Design review of the part built by this model. Coordinates are the model's own, in mm. A direction names the side the tool comes from. Coordinates: 2 decimals unless noted, no trailing zeros. Order: outer loops, then holes, each group sorted by start corner. A loop starts at its lowest first (then second) coordinate and runs counter-clockwise, first axis right, second up. Notation, with made-up numbers: M 16.5,-31 L 31.5,-31 A16 cw 31.5,-1 Z; hole C 73.25,25.5 d8. An arc over 180 degrees is marked long. Answer as a JSON object with one key per item and string values.
from build123d import *


with BuildPart() as part:
    # Sketch1 → Revolve1 (revolve)
    with BuildSketch(Plane.XY, mode=Mode.PRIVATE) as revolve1_sk:
        Polygon((-20, 7), (-20, 5), (20, 5), (20, 6), (-15, 6), (-15, 5.9), (-16, 5.9), (-16, 7), align=None)
    revolve(revolve1_sk.sketch.rotate(Axis((20, 0, 0), (-1, 0, 0)), 270), axis=Axis((20, 0, 0), (-1, 0, 0)))


solid = part.part
1) Insertion check: pin 1 Ø1 at (y, z) = (4.5, -1) entering from -X; pin 2 Ø2 at (x, z) = (-1.5, -4) entering from +Y; pin 3 Ø6 at (x, y) = (11.5, 3.5) entering from +Z; pin 4 Ø1.5 at (x, y) = (-0.5, -2.5) entering from -Z. Each pin has a flat end and moves straight along its axis. Give the tip position at first contact, or say it passes through.
Taken from the geometry:
{"pin 1": "stops at x = -20", "pin 2": "stops at y = 5.2", "pin 3": "stops at z = 5.98", "pin 4": "stops at z = -5.74"}
2) Add section C-C (z = 5.5). State the section outline as (x, y) points, and give its area (3 significant figures).
Taken from the geometry:
{"outline": "M -20,-4.33 L -16,-4.33 L -16,-2.14 L -15,-2.14 L -15,-2.4 L 20,-2.4 L 20,2.4 L -15,2.4 L -15,2.14 L -16,2.14 L -16,4.33 L -20,4.33 Z", "area": "207 mm2"}
3) Add section B-B (y = 2.75). State the section outline as (x, z) points.
Taken from the geometry:
{"outline": "M -20,-6.44 L -16,-6.44 L -16,-5.22 L -15,-5.22 L -15,-5.33 L 20,-5.33 L 20,-4.18 L -20,-4.18 Z; M -20,4.18 L 20,4.18 L 20,5.33 L -15,5.33 L -15,5.22 L -16,5.22 L -16,6.44 L -20,6.44 Z"}
4) Mouldability with a two-part tool opening along X and no side actions: class faces 3 (the cylindrical face through (-15.51, -5.76, -1.28)), 4 (the flat face through (20, 4, 4)), 5 (the flat face through (-20, 5, -2)), 6 (the cylindrical face through (-18.028, -6.834, -1.517)) as released by +X, released by -X, zero draft, split by the parting line, or undercut.
Taken from the geometry:
{"face 3": "undercut", "face 4": "released by +X", "face 5": "released by -X", "face 6": "zero draft"}
5) To check wall thickness, follow L1, parallel to Y at x = -3, z = 0; L2, parallel to Z at x = 12, y = 3; L3, parallel to Z at x = -14, y = 2.25. State the ranges of each line that lie inside material, in increasing order.
Taken from the geometry:
{"L1": "y = -6 to -5, 5 to 6", "L2": "z = -5.2 to -4, 4 to 5.2", "L3": "z = -5.56 to -4.47, 4.47 to 5.56"}
6) Add section D-D (x = -15.5). State the section outline as (y, z) points.
Taken from the geometry:
{"outline": "C 0,0 d11.8; hole C 0,0 d10"}
7) Tool access review of faces 1 (the cylindrical face through (0.28, -4.88, -1.08)), 2 (the cylindrical face through (2.255, 1.802, 5.723)): name each direction out of +Z, -Z, +X, -X, +Y, -Y from which nothing blocks a thin tool from reaching the whole face with its end or side.
Taken from the geometry:
{"face 1": "+X, -X", "face 2": "+X"}
8) Add section A-A (z = 0). State the section outline as (x, y) points, and give its area (3 significant figures).
Taken from the geometry:
{"outline": "M -20,-7 L -16,-7 L -16,-5.9 L -15,-5.9 L -15,-6 L 20,-6 L 20,-5 L -20,-5 Z; M -20,5 L 20,5 L 20,6 L -15,6 L -15,5.9 L -16,5.9 L -16,7 L -20,7 Z", "area": "87.8 mm2"}
